from build123d import *

# Parameters (mm, degrees)
CHAMFER1_SIZE = 0.5


with BuildPart() as part:
    # Sketch1 → Revolve1 (revolve)
    with BuildSketch(Plane.XY, mode=Mode.PRIVATE) as revolve1_sk:
        Polygon((88.713048819, -48.25), (88.713048819, -41.75), (90.463048819, -41.75), (90.463048819, -36.25), (92.463048819, -36.25), (92.463048819, -33.25), (82.463048819, -33.25), (82.463048819, -48.25), align=None)
    revolve(revolve1_sk.sketch.rotate(Axis((82.463048819, -48.25, 0), (0, 1, 0)), 90), axis=Axis((82.463048819, -48.25, 0), (0, 1, 0)))

    # Chamfer1
    chamfer1_edges = [part.edges().sort_by_distance(p)[0] for p in [
        (82.463048819, -33.25, 10),
        (82.463048819, -36.25, 10),
        (82.463048819, -41.75, 8),
        (82.463048819, -48.25, 6.25),
    ]]
    chamfer(chamfer1_edges, length=CHAMFER1_SIZE)


solid = part.part
Work out the finished part from the listing and answer in its coordinate system (mm). A direction names the side the tool comes from. Round coordinates to 2 decimals unless told otherwise and drop trailing zeros. Loops run counter-clockwise (first coordinate to the right, second up) from the corner with the lowest first, then second, coordinate; pieces in that order, holes last. Notation, with made-up numbers: (32.5, 4) - (84.5, 4) arc R9 ccw to (84.5, 15) - close; hole circle Ø8 at (23, 65.25). An arc over 180 degrees is marked (long way). Use one line per item in the form item = value. Start each with the question number.
(1) Flat-ended cylindrical pins translate along their axes: P1, Ø8, axis at y = -38.5, z = -3.5, coming from the +X side; P2, Ø2, axis at x = 82, y = -40.5, coming from the +Z side; P3, Ø6, axis at y = -42, z = -1, coming from the -X side. Find the tip coordinate at first contact, or state that the pin passes through.
(2) Consider line 1 (Y direction, x = 87, z = -5); line 2 (Y direction, x = 75.5, z = -5); line 3 (Z direction, x = 82.5, y = -44.75). Determine where each line is inside the solid, lowest interval first.
(3) Find section A-A on z = 0. Determine the outline of the cut face in (x, y).
(4) Find section B-B on y = -40. Determine the outline of the cut face in (x, z).
(5) Which of the six approach directions +Z, -Z, +X, -X, +Y, -Y give full straight-line access (tool end or side, diameter ignored) to faces 1 (the face through (90.273, -38.715, 1.734)), 2 (the face through (82, -48.25, 0))?
Answer list:
q1.P1 = 92.45
q1.P2 = 8
q1.P3 = 74.46
q2.line_1 = -41.75 to -33.25
q2.line_2 = -36.25 to -33.25
q2.line_3 = -6.25 to 6.25
q3.outline = (72.46, -35.75) - (72.96, -36.25) - (74.46, -36.25) - (74.46, -41.25) - (74.96, -41.75) - (76.21, -41.75) - (76.21, -47.75) - (76.71, -48.25) - (88.21, -48.25) - (88.71, -47.75) - (88.71, -41.75) - (89.96, -41.75) - (90.46, -41.25) - (90.46, -36.25) - (91.96, -36.25) - (92.46, -35.75) - (92.46, -33.75) - (91.96, -33.25) - (72.96, -33.25) - (72.46, -33.75) - close
q4.outline = circle Ø16 at (82.46, 0)
q5.face_1 = -Y
q5.face_2 = +Z, -Z, +X, -X, -Y
